Geometry check sheet. Reference: the model listing, model coordinates, mm. Face numbers are marked on the shaded views. A direction names the side the tool comes from. Coordinates: 2 decimals unless noted, no trailing zeros. Order: outer loops, then holes, each group sorted by start corner. A loop starts at its lowest first (then second) coordinate and runs counter-clockwise, first axis right, second up. Notation, with made-up numbers: (10, 12) -> (50, 12) arc R26 ccw to (50, 49) -> close; hole circle Ø7 at (14.25, -30.5). An arc over 180 degrees is marked (long way). Answer as CSV lines item,"result". Start each with the question number.
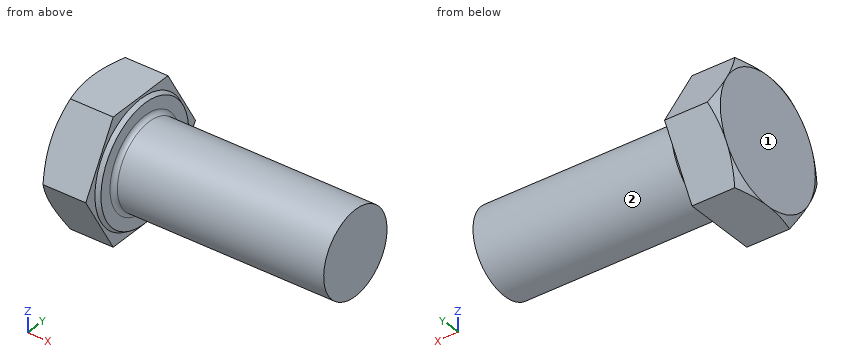
from build123d import *

# Parameters (mm, degrees)
EXTRUDE_387_DEPTH = 7.5
FILLET_1280_R     = 0.6


with BuildPart() as part:
    # 草图1 → Extrude 387 (new body)
    with BuildSketch(Plane(origin=(0, 0, 0), x_dir=(0, 0, -1), z_dir=(1, 0, 0))):
        Polygon((9, 5.196152423), (9, -5.196152423), (0, -10.392304845), (-9, -5.196152423), (-9, 5.196152423), (0, 10.392304845), align=None)
    extrude(amount=EXTRUDE_387_DEPTH)

    # 草图2 → 凸台-旋转1 (revolve)
    with BuildSketch(Plane.XY, mode=Mode.PRIVATE) as revolve_1_sk:
        Polygon((0, 0), (37.5, 0), (37.5, 4.4845), (37.5, 6), (7.5, 6), (0, 6), align=None)
    revolve(revolve_1_sk.sketch.rotate(Axis((0, 0, 0), (1, 0, 0)), 90), axis=Axis((0, 0, 0), (1, 0, 0)))

    # 草图3 → 切除-旋转1 (revolve, cut)
    with BuildSketch(Plane.XY):
        Polygon((0, 9), (3.690598923, 15.392304845), (3.690598923, 20.392304845), (-10, 20.392304845), (-10, 9), align=None)
    revolve(axis=Axis((0, 0, 0), (1, 0, 0)), mode=Mode.SUBTRACT)

    # 草图4 → 切除-旋转3 (revolve, cut)
    with BuildSketch(Plane.XY, mode=Mode.PRIVATE) as cut_revolve_3_sk:
        Polygon((7.5, 8.315), (6.9, 8.661410162), (6.9, 10.392304845), (7.5, 10.392304845), align=None)
    revolve(cut_revolve_3_sk.sketch.rotate(Axis((0, 0, 0), (1, 0, 0)), 90), axis=Axis((0, 0, 0), (1, 0, 0)), mode=Mode.SUBTRACT)

    # Fillet 1280
    fillet_1280_edges = [part.edges().sort_by_distance(p)[0] for p in [
        (7.5, 0, -6),
    ]]
    fillet(fillet_1280_edges, radius=FILLET_1280_R)


solid = part.part
Q1. Access from +Z, -Z, +X, -X, +Y, -Y to the whole of each face (thin tool, end or side, straight path). Record for the marked faces 1 and 2.
Q2. Go/stop test with flat-tipped pins: pin 1 Ø1 at (x, z) = (17, -5) entering from -Y; pin 2 Ø2 at (x, z) = (30, -1.5) entering from -Y; pin 3 Ø10 at (x, y) = (19, -5) entering from +Z. Record where each tip stops, or that it passes through.
Q3. Sectioned sample at A-A, the plane x = 30.5. Record the cut outline in (y, z), then the cut area to 3 significant figures.
Q4. Thickness scan on L1, parallel to X at y = -6.25, z = -2.25; L2, parallel to Z at x = 34, y = 0.25; L3, parallel to Y at x = 23, z = 4.25. Record the ranges inside material, lowest first.
Geometry results:
1,face 1,"+Z, -Z, -X, +Y, -Y"
1,face 2,"+X"
2,pin 1,"stops at y = -3.97"
2,pin 2,"stops at y = -5.98"
2,pin 3,"stops at z = 6"
3,outline,"circle Ø12 at (0, 0)"
3,area,"113 mm^2"
4,L1,"x = 0 to 7.5"
4,L2,"z = -5.99 to 5.99"
4,L3,"y = -4.24 to 4.24"
